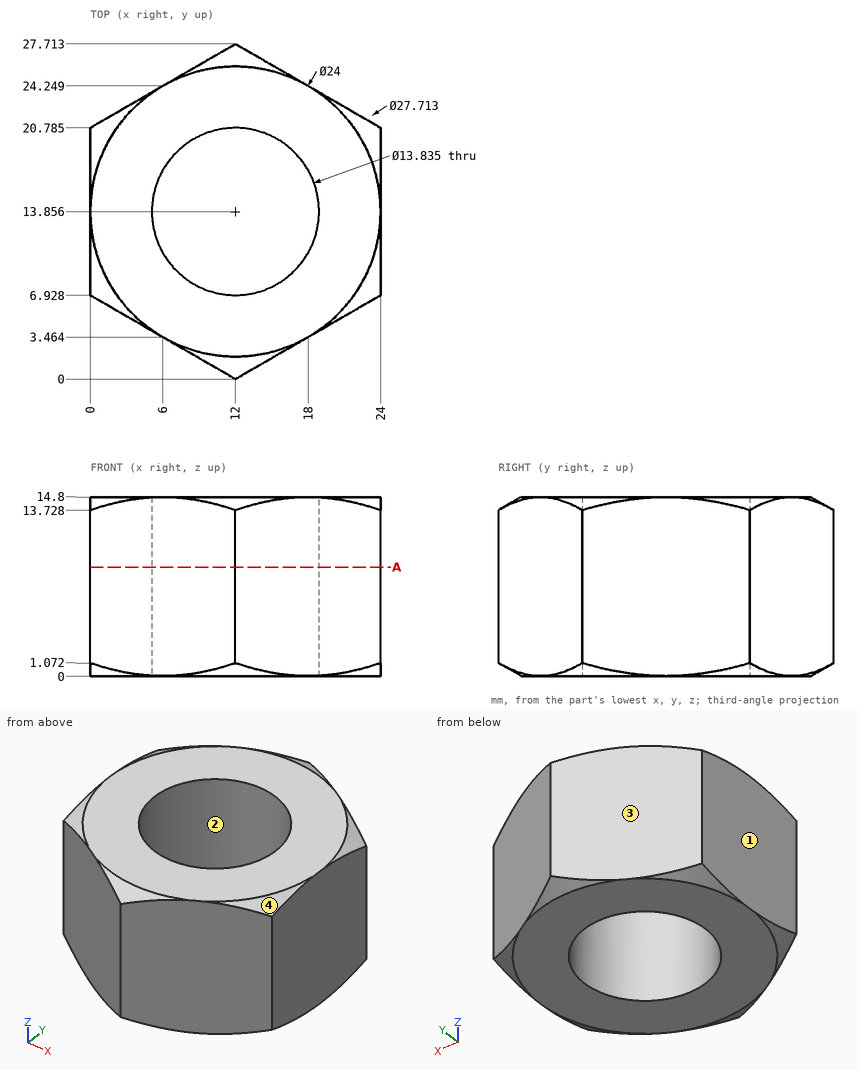
Geometry check sheet. Reference: drawing and pictorial views, mm from the part's lowest x, y, z. Coordinates: 2 decimals unless noted, no trailing zeros. Order: outer loops, then holes, each group sorted by start corner. A loop starts at its lowest first (then second) coordinate and runs counter-clockwise, first axis right, second up. Notation, with made-up numbers: (48.25, -24.5) - (68.25, -24.5) arc R25 cw to (68.25, 1.5) - close; hole circle Ø9 at (67.25, 13). An arc over 180 degrees is marked (long way). Answer in a Markdown table with one row per item. Add a question column.
1) Gauge pin test, flat ends, axial feed: P1, Ø5, axis at x = 5, z = 5.5, coming from the -Y side; P2, Ø1.5, axis at x = 17, z = 11, coming from the +Y side; P3, Ø3, axis at x = 14.5, z = 2.5, coming from the +Y side (1 decimal). Record the tip position at first contact, or that the pin passes through.
2) Cross-section at A-A, the plane z = 9. Record the cut outline in (x, y) (1 decimal).
3) Release check for a two-part mould opening along Y. For the marked faces 1, 2, 3 and 4 record: +Y half, -Y half, draft (parallel to the pull), parting line (faces both ways), or undercut.
4) Material ranges on line 1 along Y through (x, z) = (17.75, 8.5) (1 decimal); line 2 along X through (y, z) = (14.5, 9.25); line 3 along X through (y, z) = (15.25, 3) (1 decimal), recorded low to high. Write a range as [from, to].
Check result:
| question | item | result |
|---|---|---|
| 1 | P1 | stops at y = 2.6 |
| 1 | P2 | stops at y = 25.26 |
| 1 | P3 | stops at y = 27.1 |
| 2 | outline | (0, 6.9) - (12, 0) - (24, 6.9) - (24, 20.8) - (12, 27.7) - (0, 20.8) - close; hole circle Ø13.8 at (12, 13.9) |
| 3 | face 1 | draft |
| 3 | face 2 | undercut |
| 3 | face 3 | +Y half |
| 3 | face 4 | -Y half |
| 4 | line 1 | y = [3.3, 10], [17.7, 24.4] |
| 4 | line 2 | x = [0, 5.11], [18.89, 24] |
| 4 | line 3 | x = [0, 5.2], [18.8, 24] |
